Verification items for the finished model (mm, model axes). Face numbers are marked on the shaded views. A direction names the side the tool comes from. Round coordinates to 2 decimals unless told otherwise and drop trailing zeros. Order: outer loops, then holes, each group sorted by start corner. A loop starts at its lowest first (then second) coordinate and runs counter-clockwise, first axis right, second up. Notation, with made-up numbers: M -9,16 L 28,16 A22 ccw 28,36 Z; hole C 2,-5.5 d2. An arc over 180 degrees is marked long. Use one line per item in the form item = value. Start each with the question number.
Item 1: Thickness scan on probe 1 along Y at (x, z) = (-5, -1.25); probe 2 along Z at (x, y) = (-1.25, 51.5); probe 3 along Y at (x, z) = (-3.5, 1). Record the ranges inside material, lowest first. Write a range as [from, to].
Item 2: Cross-section at A-A on y = 52. Enter the section's corners in (x, z).
Item 3: Tool access check on the marked faces 1, 2, 3 and 4. Record the directions out of +Z, -Z, +X, -X, +Y, -Y that give a thin tool (end or side, any length) a straight path to the whole face; none if there is none.
Item 4: Go/stop test with flat-tipped pins: pin 1 Ø1.5 at (y, z) = (23.5, -3.5) entering from +X; pin 2 Ø1 at (x, y) = (2, 11) entering from -Z; pin 3 Ø5 at (x, y) = (-2.5, 29.5) entering from +Z; pin 4 Ø5 at (x, z) = (-2.5, -4) entering from -Y. Record where each tip stops, or that it passes through.
Item 5: Cross-section at B-B on y = 28.5. Enter the section's corners in (x, z), then the cut area to 3 significant figures.
from build123d import *

# Parameters (mm, degrees)
SKETCH1_R           = 4
BOSS_EXTRUDE1_DEPTH = 43
SKETCH2_R           = 6
BOSS_EXTRUDE2_DEPTH = 2
SKETCH10_R          = 4
BOSS_EXTRUDE4_DEPTH = 12
SKETCH8_W           = 4.085685727
SKETCH8_H           = 24
SKETCH8_W_2         = 3.929787065
SKETCH8_H_2         = 1
SKETCH9_R           = 3
BOSS_EXTRUDE3_DEPTH = 12
CHAMFER1_SIZE       = 0.2


with BuildPart() as part:
    # Sketch1 → Boss-Extrude1 (new body)
    with BuildSketch(Plane(origin=(0, 0, 0), x_dir=(1, 0, 0), z_dir=(0, 1, 0))):
        with Locations(Location((0, 0, 0), (0, 0, 270))):
            Circle(SKETCH1_R)
    extrude(amount=BOSS_EXTRUDE1_DEPTH)

    # Sketch2 → Boss-Extrude2 (add)
    with BuildSketch(Plane(origin=(0, 43, 0), x_dir=(1, 0, 0), z_dir=(0, 1, 0))):
        with Locations(Location((0, 0, 0), (0, 0, 270))):
            Circle(SKETCH2_R)
    extrude(amount=BOSS_EXTRUDE2_DEPTH)

    # Sketch10 → Boss-Extrude4 (add)
    with BuildSketch(Plane(origin=(0, 45, 0), x_dir=(1, 0, 0), z_dir=(0, 1, 0))):
        with Locations(Location((0, 0, 0), (0, 0, 270))):
            Circle(SKETCH10_R)
    extrude(amount=BOSS_EXTRUDE4_DEPTH)

    # Sketch8 → Cut-Revolve1 (revolve, cut)
    with BuildSketch(Plane.XY):
        with Locations((5.842842864, 25)):
            Rectangle(SKETCH8_W, SKETCH8_H)
        with Locations((5.214893532, 7)):
            Rectangle(SKETCH8_W_2, SKETCH8_H_2)
    revolve(axis=Axis((0, 0, 0), (0, 1, 0)), mode=Mode.SUBTRACT)

    # Sketch9 → Boss-Extrude3 (add)
    with BuildSketch(Plane.XZ):
        with Locations(Location((0, 0, 0), (0, 0, 90))):
            Circle(SKETCH9_R)
    extrude(amount=BOSS_EXTRUDE3_DEPTH)

    # Chamfer1
    chamfer1_edges = [part.edges().sort_by_distance(p)[0] for p in [
        (0, 57, -4),
        (0, 0, -4),
        (0, -12, -3),
        (0, 43, -6),
        (0, 45, -6),
    ]]
    chamfer(chamfer1_edges, length=CHAMFER1_SIZE)


solid = part.part
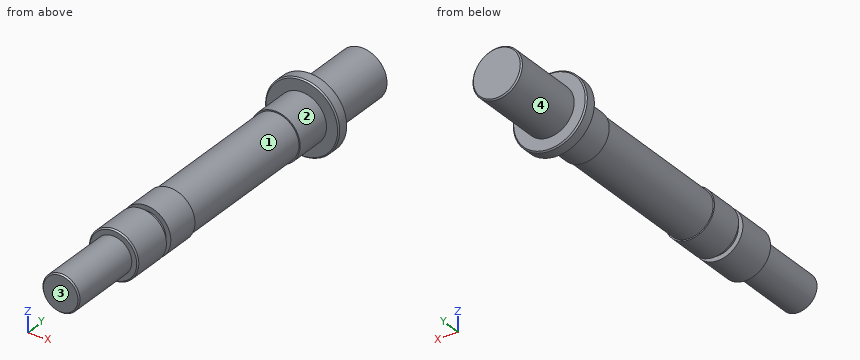
Output values:
q1.probe_1 = [43, 45]
q1.probe_2 = [-3.8, 3.8]
q1.probe_3 = [0, 6.5], [7.5, 57]
q2.outline = C 0,0 d8
q3.face_1 = none
q3.face_2 = -Y
q3.face_3 = +Z, -Z, +X, -X, -Y
q3.face_4 = +Y
q4.pin_1 = 2.62
q4.pin_2 = -3.71
q4.pin_3 = 3.8
q4.pin_4 = -12
q5.outline = C 0,0 d7.6
q5.area = 45.4 mm2
